```python
from build123d import *

# Parameters (mm, degrees)
SKETCH1_R           = 9.65
SKETCH2_R           = 9.5
SKETCH3_R           = 9.36
BOSS_EXTRUDE1_DEPTH = 3
SKETCH4_R           = 9.25
BOSS_EXTRUDE2_DEPTH = 0.2
SKETCH5_R           = 8.75
CUT_EXTRUDE1_DEPTH  = 10.2
BOSS_EXTRUDE3_START = 3
BOSS_EXTRUDE3_DEPTH = 3
CIRPATTERN1_COUNT   = 8
SKETCH8_R           = 9.25
BOSS_EXTRUDE4_DEPTH = 1
SKETCH9_R           = 9.4
BOSS_EXTRUDE5_DEPTH = 2
SKETCH11_R          = 8.75
CUT_EXTRUDE2_DEPTH  = 9


with BuildPart() as part:
    # Sketch1 → Loft2 section 0
    with BuildSketch(Plane.XY):
        Circle(SKETCH1_R)
    # Sketch2 → Loft2 section 1
    with BuildSketch(Plane.XY.offset(1.3)):
        Circle(SKETCH2_R)
    loft()

    # Sketch3 → Boss-Extrude1 (add)
    with BuildSketch(Plane.XY.offset(1.3)):
        Circle(SKETCH3_R)
    extrude(amount=BOSS_EXTRUDE1_DEPTH)

    # Sketch4 → Boss-Extrude2 (add)
    with BuildSketch(Plane.XY.offset(4.3)):
        Circle(SKETCH4_R)
    extrude(amount=BOSS_EXTRUDE2_DEPTH)

    # Sketch5 → Cut-Extrude1 (cut)
    with BuildSketch(Plane.XY.offset(4.5)):
        Circle(SKETCH5_R)
    extrude(amount=-CUT_EXTRUDE1_DEPTH, mode=Mode.SUBTRACT)

    # Sketch7 → Boss-Extrude3 (add)
    with BuildSketch(Plane.XY.offset(4.5).offset(BOSS_EXTRUDE3_START)):
        with BuildLine():
            Line((-1.666819903, 8.589773653), (-1.726800204, 8.898875558))
            ThreePointArc((-1.726800204, 8.898875558), (-0.155292705, 9.063537352), (1.420933285, 8.952808149))
            Line((1.420933285, 8.952808149), (1.371577253, 8.641832898))
            ThreePointArc((1.371577253, 8.641832898), (-0.149898622, 8.748715929), (-1.666819903, 8.589773653))
        make_face()
    boss_extrude3 = extrude(amount=-BOSS_EXTRUDE3_DEPTH)

    # CirPattern1: Boss-Extrude3 ×8 about axis
    cirpattern1_axis = Axis((0, 0, 0), (0, 0, 1))
    for i in range(1, CIRPATTERN1_COUNT):
        add(boss_extrude3.rotate(cirpattern1_axis, i * 360 / CIRPATTERN1_COUNT))

    # Sketch8 → Boss-Extrude4 (add)
    with BuildSketch(Plane.XY.offset(7.5)):
        Circle(SKETCH8_R)
    extrude(amount=BOSS_EXTRUDE4_DEPTH)

    # Sketch9 → Boss-Extrude5 (add)
    with BuildSketch(Plane.XY.offset(8.5)):
        Circle(SKETCH9_R)
    extrude(amount=BOSS_EXTRUDE5_DEPTH)

    # Sketch11 → Cut-Extrude2 (cut)
    with BuildSketch(Plane.XY.offset(10.5)):
        Circle(SKETCH11_R)
    extrude(amount=-CUT_EXTRUDE2_DEPTH, mode=Mode.SUBTRACT)


solid = part.part
```
The listing builds one solid part. Answer for the finished solid, in the listing's coordinates (mm). A direction names the side the tool comes from. Round coordinates to 2 decimals unless told otherwise and drop trailing zeros. Loops run counter-clockwise (first coordinate to the right, second up) from the corner with the lowest first, then second, coordinate; pieces in that order, holes last. Notation, with made-up numbers: (-29, 25.5) - (-9, 25.5) arc R25 ccw to (-9, 46.5) - close; hole circle Ø5 at (40.25, 27.25). An arc over 180 degrees is marked (long way). Use one line per item in the form item = value. Start each with the question number.
1. Consider line 1 (Y direction, x = 0, z = 2.7); line 2 (Z direction, x = 1.75, y = 9); line 3 (X direction, y = 7, z = 5). Determine where each line is inside the solid, lowest interval first. Write a range as [from, to].
2. A tool of negligible diameter and unlimited length cuts with its end or side. For faces 4 (the face through (-6.283, -6.534, 6.021)), 5 (the face through (6.534, -6.283, 6.021)), 6 (the face through (9.063, 0.177, 6.021)), 7 (the face through (4.8, -7.5, 7.5)), from which of +Z, -Z, +X, -X, +Y, -Y can it reach the whole face along a straight path? Write none if from no direction.
3. For a pull along Z with two mould halves and no side action, classify faces 1 (the face through (2, -9, 0)), 2 (the face through (-2.038, -9.176, 9.486)), 3 (the face through (-0.177, 9.063, 6.021)) as pulls with the +Z half, pulls with the -Z half, needs draft (parallel to the pull), parting line crosses it, or undercut.
4. Given pin 1 Ø4 at (x, z) = (-3, 7.5) entering from +Y; pin 2 Ø5 at (y, z) = (6, 9) entering from -X; pin 3 Ø1.5 at (y, z) = (7, 2.5) entering from -X, each flat-ended and moving along its own axis, determine where each tip first touches the part or whether it passes through.
5. The part is cut by section A-A on z = 7.25. Give the number of separate pieces and of enclosed holes in the cut face, then the cut area to 3 significant figures.
6. The part is cut by section B-B on x = 0. Determine the outline of the cut face in (y, z), then the cut area to 3 significant figures.
Geometry check:
q1.line_1 = [-9.36, -8.75], [8.75, 9.36]
q1.line_2 = [0, 4.5], [7.5, 10.5]
q1.line_3 = [-5.76, -5.25], [5.25, 5.76]
q2.face_4 = -X, -Y
q2.face_5 = +X, -Y
q2.face_6 = +X
q2.face_7 = none
q3.face_1 = pulls with the -Z half
q3.face_2 = needs draft
q3.face_3 = undercut
q4.pin_1 = 9.31
q4.pin_2 = -8.72
q4.pin_3 = -6.97
q5.separate_pieces = 8
q5.enclosed_holes = 0
q5.area = 7.83 mm^2
q6.outline = (-9.65, 0) - (-8.75, 0) - (-8.75, 10.5) - (-9.4, 10.5) - (-9.4, 8.5) - (-9.25, 8.5) - (-9.25, 7.5) - (-9.06, 7.5) - (-9.06, 4.5) - (-9.25, 4.5) - (-9.25, 4.3) - (-9.36, 4.3) - (-9.36, 1.3) - (-9.5, 1.3) - close; (8.75, 0) - (9.65, 0) - (9.5, 1.3) - (9.36, 1.3) - (9.36, 4.3) - (9.25, 4.3) - (9.25, 4.5) - (9.06, 4.5) - (9.06, 7.5) - (9.25, 7.5) - (9.25, 8.5) - (9.4, 8.5) - (9.4, 10.5) - (8.75, 10.5) - close
q6.area = 11.5 mm^2
